Geometry check sheet. Reference: the model listing, model coordinates, mm. Face numbers are marked on the shaded views. A direction names the side the tool comes from. Coordinates: 2 decimals unless noted, no trailing zeros. Write each loop counter-clockwise with the first axis right and the second up, starting at its lowest first coordinate (ties: lowest second). Pieces come first, ordered by that corner, then holes. Notation, with made-up numbers: (51, -18) -> (108, -18) arc R23 ccw to (108, -3) -> close; hole circle Ø10 at (30.25, -5.75). An arc over 180 degrees is marked (long way). Use a Markdown table: item, result.
```python
from build123d import *

# Parameters (mm, degrees)
SKETCH1_W           = 69
SKETCH1_H           = 60
BOSS_EXTRUDE1_DEPTH = 3
SKETCH2_W           = 6
SKETCH2_H           = 60
BOSS_EXTRUDE2_DEPTH = 24
CHAMFER1_SIZE       = 5
SKETCH3_R           = 4.25
CUT_EXTRUDE1_DEPTH  = 52.635743434
FILLET1_R           = 5
SKETCH4_R           = 3.25
CUT_EXTRUDE2_DEPTH  = 75.81978348


with BuildPart() as part:
    # Sketch1 → Boss-Extrude1 (new, symmetric)
    with BuildSketch(Plane.XY):
        Rectangle(SKETCH1_W, SKETCH1_H)
    extrude(amount=BOSS_EXTRUDE1_DEPTH, both=True)

    # Sketch2 → Boss-Extrude2 (add)
    with BuildSketch(Plane.XY.offset(3)):
        with Locations((31.5, 0)):
            Rectangle(SKETCH2_W, SKETCH2_H)
    extrude(amount=BOSS_EXTRUDE2_DEPTH)

    # Chamfer1
    chamfer1_edges = [part.edges().sort_by_distance(p)[0] for p in [
        (31.5, 30, 27),
        (31.5, -30, 27),
        (-34.5, 30, 0),
        (-34.5, -30, 0),
    ]]
    chamfer(chamfer1_edges, length=CHAMFER1_SIZE)

    # Sketch3 → Cut-Extrude1 (cut, through all)
    with BuildSketch(Plane.XY.offset(3)):
        with Locations((-14.5, 0)):
            Circle(SKETCH3_R)
        with Locations((0.5, 0)):
            Circle(SKETCH3_R)
    extrude(amount=-CUT_EXTRUDE1_DEPTH, mode=Mode.SUBTRACT)

    # Fillet1
    fillet1_edges = [part.edges().sort_by_distance(p)[0] for p in [
        (28.5, 0, 3),
    ]]
    fillet(fillet1_edges, radius=FILLET1_R)

    # Sketch4 → Cut-Extrude2 (cut, through all)
    with BuildSketch(Plane.ZY.offset(-28.5)):
        with Locations(Location((17, 20, 0), (0, 0, 270))):
            Circle(SKETCH4_R)
        with Locations(Location((17, -20, 0), (0, 0, 270))):
            Circle(SKETCH4_R)
    extrude(amount=-CUT_EXTRUDE2_DEPTH, mode=Mode.SUBTRACT)


solid = part.part
```
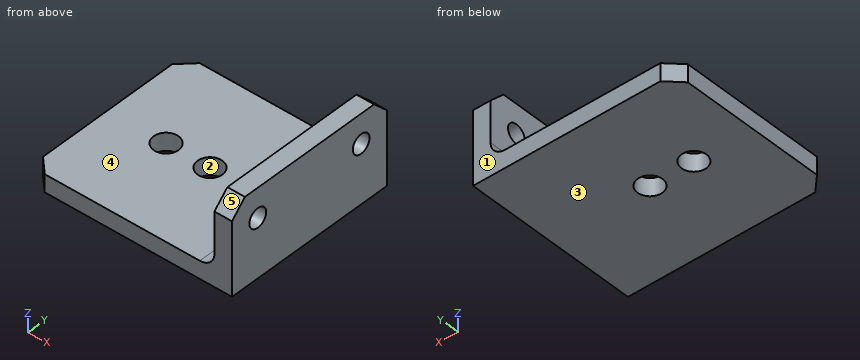
Item 1: Tool access check on the marked faces 4 and 5. Record the directions out of +Z, -Z, +X, -X, +Y, -Y that give a thin tool (end or side, any length) a straight path to the whole face; none if there is none.
Answer block:
| item | result |
|---|---|
| face 4 | +Z, -X, +Y, -Y |
| face 5 | +Z, +X, -X, -Y |
Item 2: Section check D-D on y = 0. Record the boundary of the cut face in (x, z).
Answer block:
| item | result |
|---|---|
| outline | (-34.5, -3) -> (-18.75, -3) -> (-18.75, 3) -> (-34.5, 3) -> close; (-10.25, -3) -> (-3.75, -3) -> (-3.75, 3) -> (-10.25, 3) -> close; (4.75, -3) -> (34.5, -3) -> (34.5, 27) -> (28.5, 27) -> (28.5, 8) arc R5 cw to (23.5, 3) -> (4.75, 3) -> close |
Item 3: Section check C-C on x = -14.5. Record the boundary of the cut face in (y, z).
Answer block:
| item | result |
|---|---|
| outline | (-30, -3) -> (-4.25, -3) -> (-4.25, 3) -> (-30, 3) -> close; (4.25, -3) -> (30, -3) -> (30, 3) -> (4.25, 3) -> close |
Item 4: Mould release check, pull along Y, two halves, no side actions. Record for the marked faces 1, 2 and 3: +Y half, -Y half, draft (parallel to the pull), parting line (faces both ways), or undercut.
Answer block:
| item | result |
|---|---|
| face 1 | +Y half |
| face 2 | undercut |
| face 3 | draft |
Item 5: Thickness scan on L1, parallel to Z at x = 32.5, y = 20; L2, parallel to Y at x = 0.5, z = 1.1; L3, parallel to Z at x = 21, y = -2.5. Record the ranges inside material, lowest first. Write a range as [from, to].
Answer block:
| item | result |
|---|---|
| L1 | z = [-3, 13.75], [20.25, 27] |
| L2 | y = [-30, -4.25], [4.25, 30] |
| L3 | z = [-3, 3] |
Item 6: Section check B-B on z = 17. Record the boundary of the cut face in (x, y), then the cut area to 3 significant figures.
Answer block:
| item | result |
|---|---|
| outline | (28.5, -30) -> (34.5, -30) -> (34.5, -23.25) -> (28.5, -23.25) -> close; (28.5, -16.75) -> (34.5, -16.75) -> (34.5, 16.75) -> (28.5, 16.75) -> close; (28.5, 23.25) -> (34.5, 23.25) -> (34.5, 30) -> (28.5, 30) -> close |
| area | 282 mm^2 |
Item 7: Depth check by flat-ended pin: P1, Ø6, axis at y = -12, z = 10, coming from the -X side; P2, Ø15, axis at y = -2, z = 20.5, coming from the -X side; P3, Ø7.5, axis at x = 0.5, y = 0, coming from the -Z side; P4, Ø17.5, axis at x = -9, y = -5.5, coming from the +Z side. Enter the tip coordinate at first touch or a pass-through.
Answer block:
| item | result |
|---|---|
| P1 | stops at x = 28.4 |
| P2 | stops at x = 28.5 |
| P3 | passes through |
| P4 | stops at z = 3 |
Item 8: Section check A-A on y = -20. Record the boundary of the cut face in (x, z).
Answer block:
| item | result |
|---|---|
| outline | (-34.5, -3) -> (34.5, -3) -> (34.5, 13.75) -> (28.5, 13.75) -> (28.5, 8) arc R5 cw to (23.5, 3) -> (-34.5, 3) -> close; (28.5, 20.25) -> (34.5, 20.25) -> (34.5, 27) -> (28.5, 27) -> close |
